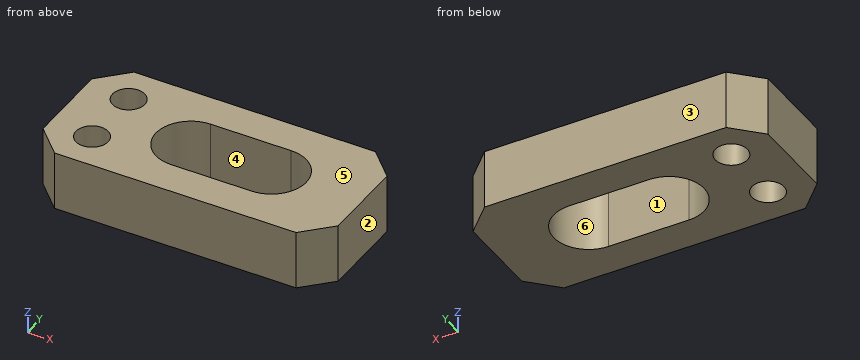
from build123d import *

# Parameters (mm, degrees)
SKETCH_1_W      = 55
SKETCH_1_H      = 26
SKETCH_1_R      = 3
EXTRUDE_1_DEPTH = 11
CHAMFER_1_SIZE  = 5


with BuildPart() as part:
    # 草图1 → 凸台-拉伸1 (new body)
    with BuildSketch(Plane.XY):
        Rectangle(SKETCH_1_W, SKETCH_1_H)
        with Locations((-19.5, 6)):
            Circle(SKETCH_1_R, mode=Mode.SUBTRACT)
        with Locations((-19.5, -6)):
            Circle(SKETCH_1_R, mode=Mode.SUBTRACT)
        with BuildLine():
            Line((-4.5, 6.5), (10.5, 6.5))
            ThreePointArc((10.5, 6.5), (17, 0), (10.5, -6.5))
            Line((10.5, -6.5), (-4.5, -6.5))
            ThreePointArc((-4.5, -6.5), (-11, 0), (-4.5, 6.5))
        make_face(mode=Mode.SUBTRACT)
    extrude(amount=EXTRUDE_1_DEPTH)

    # 倒角1
    chamfer_1_edges = [part.edges().sort_by_distance(p)[0] for p in [
        (27.5, -13, 5.5),
        (-27.5, -13, 5.5),
        (-27.5, 13, 5.5),
        (27.5, 13, 5.5),
    ]]
    chamfer(chamfer_1_edges, length=CHAMFER_1_SIZE)


solid = part.part
Could you check a few things on this model? Use its own coordinates, in mm. Face numbers are marked on the shaded views. A direction names the side the tool comes from. Give positions to 0.01 mm unless a question says otherwise; leave off trailing zeros. Write each loop counter-clockwise with the first axis right and the second up, starting at its lowest first coordinate (ties: lowest second). Pieces come first, ordered by that corner, then holes. Notation, with made-up numbers: (2, 1.25) -> (10, 1.25) arc R24 cw to (10, 27.25) -> close; hole circle Ø3 at (73.5, 3). An arc over 180 degrees is marked (long way). Answer as CSV lines item,"result". Start each with the question number.
(1) If we section it at C-C, the plane z = 10: Write out the boundary of the cut face in (x, y).
(2) If we section it at B-B, the plane y = 6: Write out the boundary of the cut face in (x, z).
(3) Please list where these lines run through material, in increasing order: line 1 (Y direction, x = -19.5, z = 4.5); line 2 (Y direction, x = -2.5, z = 2.25); line 3 (X direction, y = 4.25, z = 7).
(4) If we section it at D-D, the plane y = -7: Write out the boundary of the cut face in (x, z), and give its area (3 significant figures).
(5) If we mould it in two halves opening along Y, with no side actions, what happens to the marked faces 3, 4, 5 and 6? For each: +Y half, -Y half, draft (parallel to the pull), parting line (faces both ways), or undercut.
(6) If we section it at A-A, the plane x = 5: Write out the boundary of the cut face in (y, z), and give its area (3 significant figures).
(7) Which directions (+Z, -Z, +X, -X, +Y, -Y) give clear straight access to the entire face, cutting with the end or side of a thin tool? Please do the marked faces 1 and 2.
(8) I'm going to push a flat-ended pin straight in: pin 1 Ø5.5 at (x, y) = (-19.5, 6) entering from +Z. Where does the tip first touch, or does it pass through?
Answer list:
1,outline,"(-27.5, -8) -> (-22.5, -13) -> (22.5, -13) -> (27.5, -8) -> (27.5, 8) -> (22.5, 13) -> (-22.5, 13) -> (-27.5, 8) -> close; hole circle Ø6 at (-19.5, -6); hole circle Ø6 at (-19.5, 6); hole (-4.5, -6.5) -> (10.5, -6.5) arc R6.5 ccw to (10.5, 6.5) -> (-4.5, 6.5) arc R6.5 ccw to start"
2,outline,"(-27.5, 0) -> (-22.5, 0) -> (-22.5, 11) -> (-27.5, 11) -> close; (-16.5, 0) -> (-7, 0) -> (-7, 11) -> (-16.5, 11) -> close; (13, 0) -> (27.5, 0) -> (27.5, 11) -> (13, 11) -> close"
3,line 1,"-13 to -9, -3 to 3, 9 to 13"
3,line 2,"-13 to -6.5, 6.5 to 13"
3,line 3,"-27.5 to -21.94, -17.06 to -9.42, 15.42 to 27.5"
4,outline,"(-27.5, 0) -> (-22.33, 0) -> (-22.33, 11) -> (-27.5, 11) -> close; (-16.67, 0) -> (27.5, 0) -> (27.5, 11) -> (-16.67, 11) -> close"
4,area,"543 mm^2"
5,face 3,"+Y half"
5,face 4,"undercut"
5,face 5,"draft"
5,face 6,"undercut"
6,outline,"(-13, 0) -> (-6.5, 0) -> (-6.5, 11) -> (-13, 11) -> close; (6.5, 0) -> (13, 0) -> (13, 11) -> (6.5, 11) -> close"
6,area,"143 mm^2"
7,face 1,"+Z, -Z"
7,face 2,"+Z, -Z, +X, +Y, -Y"
8,pin 1,"through"
